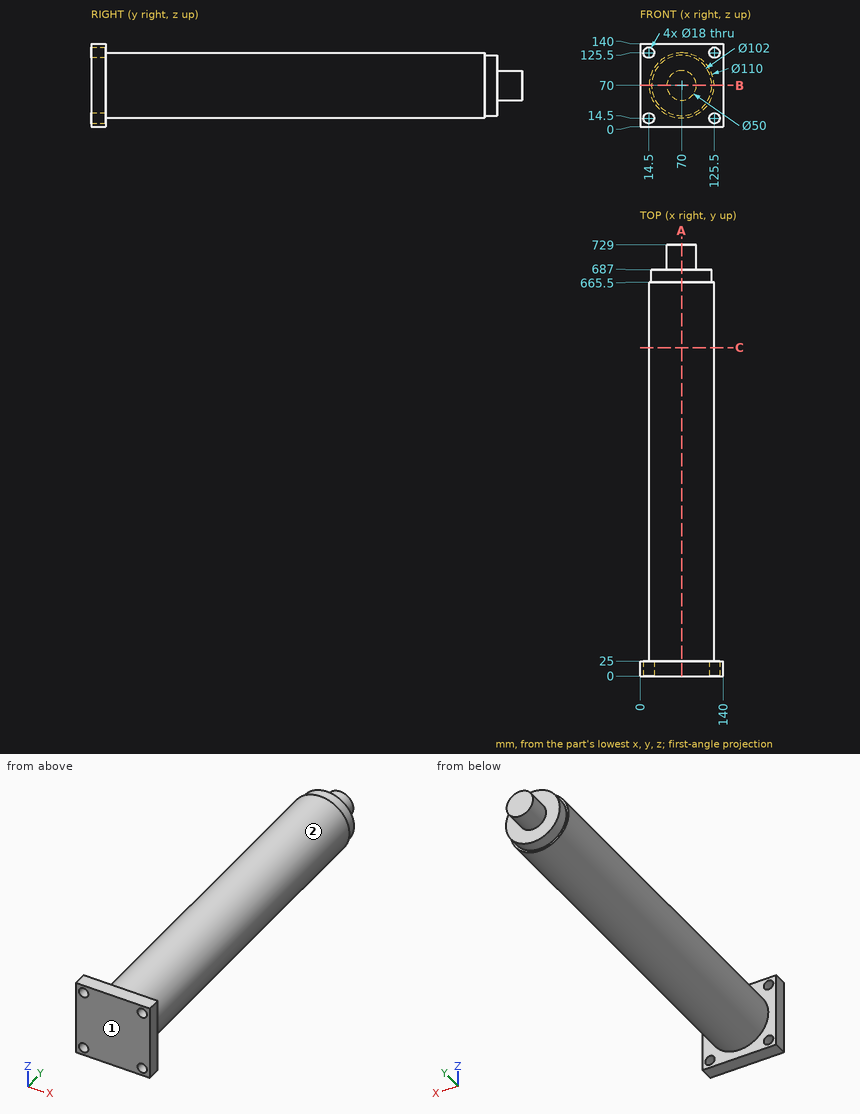
Drawing for the job (mm, zero at the part's lowest x, y, z). A direction names the side the tool comes from. Coordinates: 2 decimals unless noted, no trailing zeros. Order: outer loops, then holes, each group sorted by start corner. A loop starts at its lowest first (then second) coordinate and runs counter-clockwise, first axis right, second up. Notation, with made-up numbers: (67, 12) - (86, 12) arc R19 cw to (86, 37) - close; hole circle Ø3 at (54.5, 5). An arc over 180 degrees is marked (long way). Use a Markdown table: item, result. Add a question column.
(1) Flat gauge pins, fed straight in: pin 1 (3 mm diameter, centred on x = 23.5, y = 445, fed in from +Z); pin 2 (4 mm diameter, centred on x = 62.5, z = 113.5, fed in from +Y); pin 3 (8 mm diameter, centred on x = 63, y = 508, fed in from +Z); pin 4 (16 mm diameter, centred on x = 125.5, z = 125.5, fed in from -Y). Where does each tip first touch, or does it go through?
(2) Saw through at C-C (y = 555). Give the cut face in (x, z), then the cut area to 3 significant figures.
(3) Drill centre lines: line 1 along Z through (x, y) = (14, 16); line 2 along X through (y, z) = (7, 14.5); line 3 along Y through (x, z) = (28.5, 89). Where is each one in solid material? Low to high. Write a range as [from, to].
(4) Saw through at A-A (x = 70). Give the cut face in (y, z).
(5) Saw through at B-B (z = 70). Give the cut face in (x, y), then the cut area to 3 significant figures.
(6) Which spindle directions (+Z, -Z, +X, -X, +Y, -Y) get a long thin tool onto all of the face, cutting with end or side? Do the marked faces 1 and 2. Say none if no direction does.
Solved:
| question | item | result |
|---|---|---|
| 1 | pin 1 | stops at z = 101.62 |
| 1 | pin 2 | stops at y = 687 |
| 1 | pin 3 | stops at z = 124.92 |
| 1 | pin 4 | passes through |
| 2 | outline | circle Ø110 at (70, 70) |
| 2 | area | 9,500 mm² |
| 3 | line 1 | z = [0, 5.51], [23.49, 116.51], [134.49, 140] |
| 3 | line 2 | x = [0, 5.5], [23.5, 116.5], [134.5, 140] |
| 3 | line 3 | y = [0, 687] |
| 4 | outline | (0, 0) - (25, 0) - (25, 15) - (665.5, 15) - (665.5, 19) - (687, 19) - (687, 45) - (729, 45) - (729, 95) - (687, 95) - (687, 121) - (665.5, 121) - (665.5, 125) - (25, 125) - (25, 140) - (0, 140) - close |
| 5 | outline | (0, 0) - (140, 0) - (140, 25) - (125, 25) - (125, 665.5) - (121, 665.5) - (121, 687) - (95, 687) - (95, 729) - (45, 729) - (45, 687) - (19, 687) - (19, 665.5) - (15, 665.5) - (15, 25) - (0, 25) - close |
| 5 | area | 78,200 mm² |
| 6 | face 1 | +Z, -Z, +X, -X, -Y |
| 6 | face 2 | +Y |
